from build123d import *

# Parameters (mm, degrees)
SLOTTED_ARM_PLATE_DEPTH   = 11
END_WALL_DEPTH            = 25
END_WALL_FILLET_R10_R     = 10
WALL_NOTCH_SKETCH_R       = 3.5
WALL_NOTCH_CUT_DEPTH      = 25
HUB_WITH_KEYED_BORE_DEPTH = 25
EYE_START                 = 12
EYE_LUG_SKETCH_R          = 4.5
EYE_LUG_DEPTH             = 12


with BuildPart() as part:
    # Slotted Arm Sketch → Slotted Arm Plate (new body)
    with BuildSketch(Plane.XY):
        with BuildLine():
            Line((-77.5, 25), (77.5, 25))
            ThreePointArc((77.5, 25), (102.5, 0), (77.5, -25))
            Line((77.5, -25), (-77.5, -25))
            Line((-77.5, -25), (-77.5, 25))
        make_face()
        with BuildLine():
            Line((52.5, 12), (77.5, 12))
            ThreePointArc((77.5, 12), (89.5, 0), (77.5, -12))
            Line((77.5, -12), (52.5, -12))
            ThreePointArc((52.5, -12), (40.5, 0), (52.5, 12))
        make_face(mode=Mode.SUBTRACT)
    extrude(amount=SLOTTED_ARM_PLATE_DEPTH)

    # End Wall Sketch → End Wall (add, symmetric)
    with BuildSketch(Plane(origin=(0, 0, 0), x_dir=(1, 0, 0), z_dir=(0, 1, 0))):
        Polygon((-77.5, 0), (-77.5, 32), (-67.5, 32), (-67.5, 16), (-62.5, 16), (-62.5, 0), align=None)
    extrude(amount=END_WALL_DEPTH, both=True)

    # End Wall Fillet R10
    end_wall_fillet_r10_edges = [part.edges().sort_by_distance(p)[0] for p in [
        (-72.5, -25, -32),
        (-72.5, 25, -32),
    ]]
    fillet(end_wall_fillet_r10_edges, radius=END_WALL_FILLET_R10_R)

    # Wall Notch Sketch → Wall Notch Cut (cut, symmetric)
    with BuildSketch(Plane.ZY.offset(77.5)):
        with Locations((-22, 15)):
            Circle(WALL_NOTCH_SKETCH_R)
        with Locations((-22, -15)):
            Circle(WALL_NOTCH_SKETCH_R)
    extrude(amount=WALL_NOTCH_CUT_DEPTH, both=True, mode=Mode.SUBTRACT)

    # Hub Sketch → Hub With Keyed Bore (add, symmetric)
    with BuildSketch(Plane(origin=(0, 0, 0), x_dir=(1, 0, 0), z_dir=(0, 1, 0))):
        with BuildLine():
            Line((18.5, 0), (18.5, 31))
            ThreePointArc((18.5, 31), (0, 49.5), (-18.5, 31))
            Line((-18.5, 31), (-18.5, 0))
            Line((-18.5, 0), (18.5, 0))
        make_face()
        with BuildLine():
            ThreePointArc((2.5, 20.287857357), (0, 42), (-2.5, 20.287857357))
            Line((-2.5, 20.287857357), (-2.5, 14))
            Line((-2.5, 14), (2.5, 14))
            Line((2.5, 14), (2.5, 20.287857357))
        make_face(mode=Mode.SUBTRACT)
    extrude(amount=HUB_WITH_KEYED_BORE_DEPTH, both=True)

    # Eye Lug Sketch → Eye Lug (add)
    with BuildSketch(Plane(origin=(0, 0, 0), x_dir=(1, 0, 0), z_dir=(0, 1, 0)).offset(EYE_START)):
        with BuildLine():
            Line((17.118883443, 38.013831311), (26.545966406, 51.477101054))
            ThreePointArc((26.545966406, 51.477101054), (24.090210327, 65.40438586), (10.16292552, 62.948629781))
            Line((10.16292552, 62.948629781), (0.735842557, 49.485360038))
            ThreePointArc((0.735842557, 49.485360038), (10.611164072, 46.154312819), (17.118883443, 38.013831311))
        make_face()
        with Locations(Location((18.354445963, 57.212865417, 0), (0, 0, 270))):
            Circle(EYE_LUG_SKETCH_R, mode=Mode.SUBTRACT)
    extrude(amount=-EYE_LUG_DEPTH)


solid = part.part
Build history of the part. All positions in model axes, mm. A direction names the side the tool comes from. Round coordinates to 2 decimals unless told otherwise and drop trailing zeros. Loops run counter-clockwise (first coordinate to the right, second up) from the corner with the lowest first, then second, coordinate; pieces in that order, holes last. Notation, with made-up numbers: (31, -38.75) -> (71, -38.75) arc R30 cw to (71, 0.25) -> close; hole circle Ø1 at (-10.75, 61.5). An arc over 180 degrees is marked (long way). One line per item, written item: value. Start each with the question number.
Q1. Cut at C-C on x = -42.5. List the corners of the cut face in (y, z), plus the area to 3 significant figures.
Q2. Cut at B-B on z = -55. List the corners of the cut face in (x, y).
Q3. Drop flat-ended pins along their axis: pin 1 Ø1.9 at (y, z) = (-1, -16) entering from +X; pin 2 Ø8 at (x, y) = (-71.5, 1) entering from -Z; pin 3 Ø5.5 at (x, y) = (0, -2) entering from -Z. Give the stop position or say it passes through.
Q4. Two-plate mould, pull along X, no slides. Class faces 1 (the face through (-72.43, -21.99, -29.15)), 2 (the face through (-65, 0, -16)), 3 (the face through (65, -12, 5)), 4 (the face through (102.494, 0.55, 5.423)): released by +X, released by -X, zero draft, split by the parting line, or undercut.
Q5. 3-axis set-ups, long thin cutter, end or side, ignore diameter. For faces 5 (the face through (21.8, 6.1, -44.7)), 6 (the face through (-72.43, 22.15, -28.99)), 7 (the face through (-2.5, 0, -17)), 8 (the face through (65, 12, 5)): which of +Z, -Z, +X, -X, +Y, -Y reach the whole face in a straight line?
Q6. Cut at A-A on y = 6.5. List the corners of the cut face in (x, z).
Q7. Probe line 1 along Y through (x, z) = (-74, -22); line 2 along X through (y, z) = (10, -31); line 3 along X through (y, z) = (15, -13). List the from-to ranges inside material, lowest first.
Computed:
1. outline: (-25, 0) -> (25, 0) -> (25, 11) -> (-25, 11) -> close
1. area: 550 mm²
2. outline: (4.6, 0) -> (14.44, 0) -> (14.44, 12) -> (4.6, 12) -> close; (22.27, 0) -> (28.11, 0) -> (28.11, 12) -> (22.27, 12) -> close
3. pin 1: x = 18.5
3. pin 2: z = -32
3. pin 3: z = -51.13
4. face 1: zero draft
4. face 2: undercut
4. face 3: undercut
4. face 4: released by +X
5. face 5: +X, +Y, -Y
5. face 6: -Z, -X, +Y
5. face 7: +Y, -Y
5. face 8: +Z, -Z
6. outline: (-77.5, -32) -> (-67.5, -32) -> (-67.5, -16) -> (-62.5, -16) -> (-62.5, 0) -> (-18.5, 0) -> (-18.5, -31) arc R18.5 ccw to (0.74, -49.49) -> (10.16, -62.95) arc R10 ccw to (26.55, -51.48) -> (17.12, -38.01) arc R18.5 ccw to (18.5, -31) -> (18.5, 0) -> (42.41, 0) -> (42.41, 11) -> (-77.5, 11) -> close; (87.59, 0) -> (101.64, 0) -> (101.64, 11) -> (87.59, 11) -> close; hole (-2.5, -20.29) arc R11 ccw (long way) to (2.5, -20.29) -> (2.5, -14) -> (-2.5, -14) -> close; hole circle Ø9 at (18.35, -57.21)
7. line 1: -25 to -18.5, -11.5 to 11.5, 18.5 to 25
7. line 2: -77.5 to -67.5, -18.5 to -11, 11 to 18.5
7. line 3: -77.5 to -62.5, -18.5 to 18.5
